Input: part model. Units: mm. Frame: model coordinates. A direction names the side the tool comes from. Round coordinates to 2 decimals unless told otherwise and drop trailing zeros. Loops run counter-clockwise (first coordinate to the right, second up) from the corner with the lowest first, then second, coordinate; pieces in that order, holes last. Notation, with made-up numbers: (39.5, 84.5) -> (89.5, 84.5) arc R18 cw to (89.5, 119.5) -> close; hole circle Ø10 at (69.5, 34). An arc over 180 degrees is marked (long way). Answer as a JSON object with one key per item and string values.
```python
from build123d import *

# Parameters (mm, degrees)
SKETCH1_W                               = 37
SKETCH1_H                               = 90
BOSS_EXTRUDE1_DEPTH                     = 4
SKETCH6_W                               = 37
SKETCH6_H                               = 34
BOSS_EXTRUDE2_DEPTH                     = 15
M3_TAPPED_HOLE1_D                       = 2.5
CBORE_FOR_M4_HEX_HEAD_BOLT1_D           = 4.5
CBORE_FOR_M4_HEX_HEAD_BOLT1_CBORE_D     = 8
CBORE_FOR_M4_HEX_HEAD_BOLT1_CBORE_DEPTH = 4.5
SKETCH7_W                               = 15
SKETCH7_H                               = 26
CUT_EXTRUDE1_DEPTH                      = 100.146356464
CUT_EXTRUDE2_REACH                      = 101.99
SKETCH8_W                               = 10
SKETCH8_H                               = 64
FILLET1_R                               = 3
CHAMFER1_SIZE                           = 1
CHAMFER2_SIZE                           = 1


with BuildPart() as part:
    # Sketch1 → Boss-Extrude1 (new, symmetric)
    with BuildSketch(Plane.XY):
        with Locations((18.5, -45)):
            Rectangle(SKETCH1_W, SKETCH1_H)
    extrude(amount=BOSS_EXTRUDE1_DEPTH, both=True)

    # Sketch6 → Boss-Extrude2 (add)
    with BuildSketch(Plane.XY.offset(-4)):
        with Locations((18.5, -17)):
            Rectangle(SKETCH6_W, SKETCH6_H)
    extrude(amount=-BOSS_EXTRUDE2_DEPTH)

    # M3 Tapped Hole1 (through all)
    with Locations(Plane.XY.offset(4)):
        with Locations((18.5, -21), (18.5, -6)):
            Hole(M3_TAPPED_HOLE1_D / 2)

    # CBORE for M4 Hex Head Bolt1 (through all)
    with Locations(Plane.XY.offset(4)):
        with Locations((6, -85), (21, -85)):
            CounterBoreHole(CBORE_FOR_M4_HEX_HEAD_BOLT1_D / 2, CBORE_FOR_M4_HEX_HEAD_BOLT1_CBORE_D / 2, CBORE_FOR_M4_HEX_HEAD_BOLT1_CBORE_DEPTH)

    # Sketch7 → Cut-Extrude1 (cut, through all)
    with BuildSketch(Plane(origin=(37, 0, 0), x_dir=(0, 0, -1), z_dir=(1, 0, 0))):
        with Locations((3.5, -13)):
            Rectangle(SKETCH7_W, SKETCH7_H)
    extrude(amount=-CUT_EXTRUDE1_DEPTH, mode=Mode.SUBTRACT)

    # Cut-Extrude2: up to this face of the body (flat: up to its plane)
    cut_extrude2_end = Plane(part.part.faces().sort_by_distance((18.5, -12.99484475, -11))[0])
    # Sketch8 → Cut-Extrude2 (cut, up to the picked face)
    with BuildSketch(Plane.XY.offset(4), mode=Mode.PRIVATE) as cut_extrude2_sk1:
        with Locations((32, -58)):
            Rectangle(SKETCH8_W, SKETCH8_H)
    cut_extrude2_tool1 = split(extrude(cut_extrude2_sk1.sketch, amount=-CUT_EXTRUDE2_REACH, mode=Mode.PRIVATE), bisect_by=cut_extrude2_end, keep=Keep.BOTH, mode=Mode.PRIVATE)
    add(cut_extrude2_tool1.solids().sort_by(Axis((32, -58, 4), (0, 0, -1)))[0], mode=Mode.SUBTRACT)

    # Fillet1
    fillet1_edges = [part.edges().sort_by_distance(p)[0] for p in [
        (13.5, -34, -4),
        (13.5, -26, -11),
    ]]
    fillet(fillet1_edges, radius=FILLET1_R)

    # Chamfer1
    chamfer1_edges = [part.edges().sort_by_distance(p)[0] for p in [
        (37, -34, -15),
        (37, 0, -15),
        (0, 0, -15),
        (0, -90, 0),
        (27, -90, 0),
    ]]
    chamfer(chamfer1_edges, length=CHAMFER1_SIZE)

    # Chamfer2
    chamfer2_edges = [part.edges().sort_by_distance(p)[0] for p in [
        (13.5, -26, 4),
        (18, -34, -19),
    ]]
    chamfer(chamfer2_edges, length=CHAMFER2_SIZE)


solid = part.part
```
1) Reachability of faces 1 (the face through (14, -26, -2)), 2 (the face through (5.133, -88.905, 1.781)), 3 (the face through (13, -63, -4)), 4 (the face through (27, -56, 0)) from +Z, -Z, +X, -X, +Y, -Y: full face, straight path, thin tool, end or side. Return the list, or none.
Output:
{"face 1": "+Z, +X, -X, +Y", "face 2": "+Z", "face 3": "-Z, +X, -X, -Y", "face 4": "+Z, +X, +Y, -Y"}
2) Section B-B, the plane y = -6. Output: boundary loops of the cut face in (x, z), plus the area to 3 significant figures.
Output:
{"outline": "(0, -19) -> (17.25, -19) -> (17.25, -11) -> (0, -11) -> close; (19.75, -19) -> (37, -19) -> (37, -11) -> (19.75, -11) -> close", "area": "276 mm^2"}
3) Section A-A, the plane x = 6. Output: boundary loops of the cut face in (y, z).
Output:
{"outline": "(-90, -4) -> (-87.25, -4) -> (-87.25, -0.5) -> (-89, -0.5) -> (-89, 4) -> (-90, 4) -> close; (-82.75, -4) -> (-37, -4) arc R3 cw to (-34, -7) -> (-34, -18) -> (-33, -19) -> (0, -19) -> (0, -11) -> (-23, -11) arc R3 cw to (-26, -8) -> (-26, 3) -> (-27, 4) -> (-81, 4) -> (-81, -0.5) -> (-82.75, -0.5) -> close"}
4) Draft query along Y for faces 5 (the face through (13, -90, 0)), 6 (the face through (20.133, -88.905, 1.781)), 7 (the face through (18, 0, -15)). Return one class per face: +Y half, -Y half, draft (parallel to the pull), parting line (faces both ways), or undercut.
Output:
{"face 5": "-Y half", "face 6": "undercut", "face 7": "+Y half"}
5) Ray query, probe 1 along Y at (x, z) = (18.5, -14.5); probe 2 along Y at (x, z) = (6, -2.85); probe 3 along Z at (x, y) = (9, -60). Return the intervals inside material, ascending.
Output:
{"probe 1": "y = -34 to -22.25, -19.75 to -7.25, -4.75 to 0", "probe 2": "y = -90 to -87.25, -82.75 to -26", "probe 3": "z = -4 to 4"}
6) Section C-C, the plane z = 1.25. Output: boundary loops of the cut face in (x, y), plus the area to 3 significant figures.
Output:
{"outline": "(0, -89) -> (1, -90) -> (26, -90) -> (27, -89) -> (27, -26) -> (0, -26) -> close; hole circle Ø8 at (6, -85); hole circle Ø8 at (21, -85)", "area": "1,630 mm^2"}
7) Contact query for flat-ended pins moving along their axis: P1, Ø2, axis at y = -27, z = -0.5, coming from the +X side; P2, Ø9, axis at x = 21, y = -85, coming from the -Z side; P3, Ø5.5, axis at x = 7.5, z = -4, coming from the +Y side; P4, Ø6.5, axis at x = 7, y = -86.5, coming from the +Z side. Output: stop coordinate, or through.
Output:
{"P1": "stops at x = 27", "P2": "stops at z = -4", "P3": "stops at y = -26", "P4": "stops at z = 4"}
8) Section D-D, the plane z = -3. Output: boundary loops of the cut face in (x, y).
Output:
{"outline": "(0, -89) -> (1, -90) -> (26, -90) -> (27, -89) -> (27, -26) -> (0, -26) -> close; hole circle Ø4.5 at (6, -85); hole circle Ø4.5 at (21, -85)"}
